Source: three-view drawing plus pictorial views. Frame: mm from the lowest corner of the part. A direction names the side the tool comes from. Give positions to 0.01 mm unless a question says otherwise; leave off trailing zeros. Write each loop counter-clockwise with the first axis right and the second up, starting at its lowest first coordinate (ties: lowest second). Pieces come first, ordered by that corner, then holes. Notation, with made-up numbers: (63, 46) -> (110, 46) arc R20 ccw to (110, 62) -> close; hole circle Ø10 at (19.5, 89). An arc over 180 degrees is marked (long way). Write item = value, one per line.
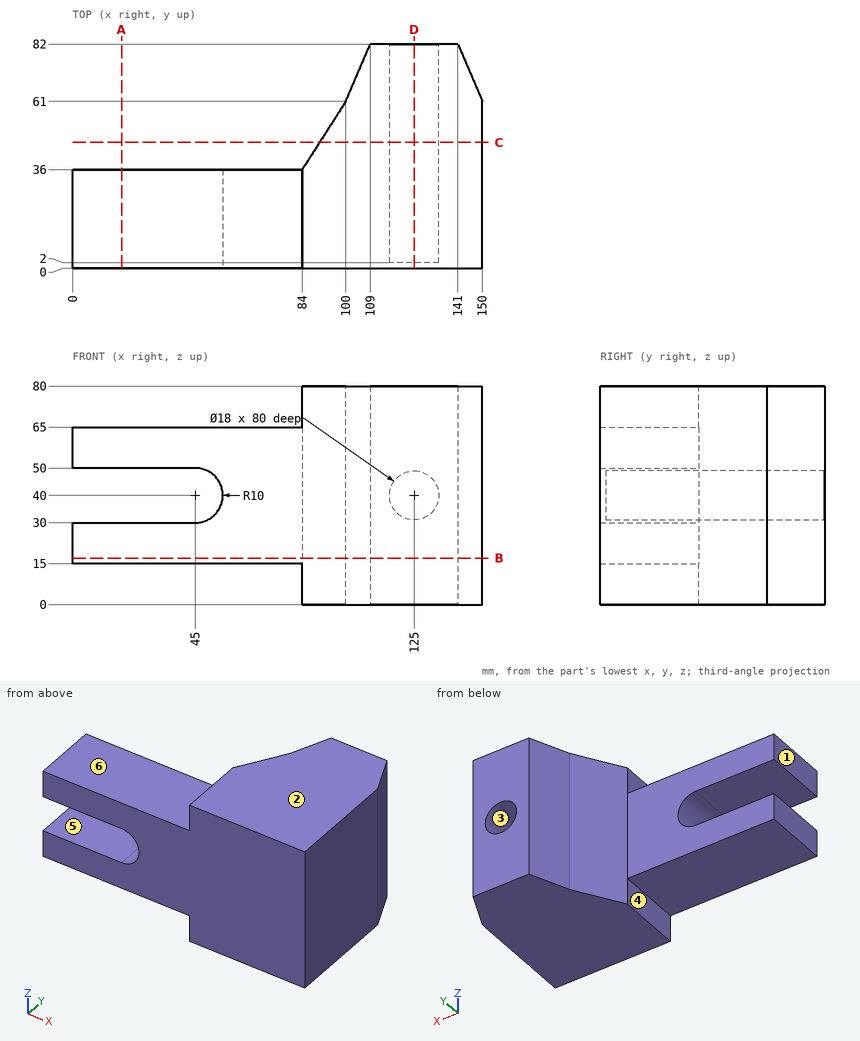
1) Cut plane B-B (z = 17). Return the cut outline in (x, y), then the cut area to 3 significant figures.
Computed:
outline = (0, 0) -> (150, 0) -> (150, 61) -> (141, 82) -> (109, 82) -> (100, 61) -> (84, 36) -> (0, 36) -> close
area = 7,710 mm²
2) Cut plane D-D (x = 125). Return the cut outline in (y, z), then the cut area to 3 significant figures.
Computed:
outline = (0, 0) -> (82, 0) -> (82, 31) -> (2, 31) -> (2, 49) -> (82, 49) -> (82, 80) -> (0, 80) -> close
area = 5,120 mm²
3) Access query for the marked faces 4, 5 and 6. Directions: +Z, -Z, +X, -X, +Y, -Y. A direction counts if a zero-diameter tool reaches every point of the face in a straight line with its end or side. Return the directions, or none.
Computed:
face_4 = -Z, -X, +Y, -Y
face_5 = -X, +Y, -Y
face_6 = +Z, -X, +Y, -Y
4) Material intervals for L1, parallel to Z at x = 19.5, y = 17; L2, parallel to X at y = 29, z = 40; L3, parallel to X at y = 8.5, z = 69.5, sorted ascending.
Computed:
L1 = 15 to 30, 50 to 65
L2 = 55 to 116, 134 to 150
L3 = 84 to 150
5) Cut plane A-A (x = 18). Return the cut outline in (y, z), then the cut area to 3 significant figures.
Computed:
outline = (0, 15) -> (36, 15) -> (36, 30) -> (0, 30) -> close; (0, 50) -> (36, 50) -> (36, 65) -> (0, 65) -> close
area = 1,080 mm²
6) Draft query along X for the marked faces 1, 2 and 3. Return one class per face: pulls with the +X half, pulls with the -X half, needs draft (parallel to the pull), parting line crosses it, or undercut.
Computed:
face_1 = pulls with the -X half
face_2 = needs draft
face_3 = undercut
7) Contact query for flat-ended pins moving along their axis: pin 1 (12 mm diameter, centred on x = 45.5, y = 25, fed in from +Z); pin 2 (5 mm diameter, centred on y = 71, z = 60, fed in from -X); pin 3 (4.5 mm diameter, centred on y = 26.5, z = 76, fed in from -X). Output: stop coordinate, or through.
Computed:
pin_1 = 65
pin_2 = 103.21
pin_3 = 84
8) Cut plane C-C (y = 46). Return the cut outline in (x, z), then the cut area to 3 significant figures.
Computed:
outline = (90.4, 0) -> (150, 0) -> (150, 80) -> (90.4, 80) -> close; hole circle Ø18 at (125, 40)
area = 4,510 mm²
